Could you check a few things on this model? Use its own coordinates, in mm. Give positions to 0.01 mm unless a question says otherwise; leave off trailing zeros. Loops run counter-clockwise (first coordinate to the right, second up) from the corner with the lowest first, then second, coordinate; pieces in that order, holes last.
1. For P1, Ø1.5, axis at x = 37, y = 8, coming from the -Z side; P2, Ø8, axis at y = 23, z = -101.5, coming from the -X side; P3, Ø6, axis at x = 19.5, y = 24, coming from the -Z side, each with a flat end and sliding along its axis, tell me the tip position at first contact or that it passes through.
2. Thinking about a two-plate mould opening in Y: for faces 1 (the flat face through (36, 30, -13)), 2 (the flat face through (36, 0, -13)), 3 (the flat face through (148, 15, -182.326)), which applies, +Y half, -Y half, draft (parallel to the pull), parting line (faces both ways), or undercut?
3. Imagine slicing it at A-A (y = 15.75). List the corners of the cut face in (x, z) for me.
4. Imagine slicing it at B-B (z = -164.5). List the corners of the cut face in (x, y) for me.
5. I need wall thicknesses on line 1 along Z through (x, y) = (-13, 4); line 2 along X through (y, z) = (24.75, -147.5); line 3 along Z through (x, y) = (19.5, 22.75). Which ranges of each line are inside material? Lowest first, please.
6. Imagine slicing it at C-C (x = -41). List the corners of the cut face in (y, z) for me, plus the area to 3 significant figures.
```python
from build123d import *

# Parameters (mm, degrees)
EXTRUDE_1_DEPTH = 30


with BuildPart() as part:
    # 草图1 → 凸台-拉伸1 (new body)
    with BuildSketch(Plane(origin=(0, 0, 0), x_dir=(1, 0, 0), z_dir=(0, 1, 0))):
        Polygon((162.790697674, 182.325581395), (132.790697674, 182.325581395), (-87.209302326, 52.325581395), (-87.209302326, -97.674418605), (162.790697674, -97.674418605), align=None)
    extrude(amount=EXTRUDE_1_DEPTH)


solid = part.part
```
Derived:
1. P1: stops at z = -126.17
1. P2: stops at x = -10.76
1. P3: stops at z = -117.15
2. face 1: +Y half
2. face 2: -Y half
2. face 3: draft
3. outline: (-87.21, -52.33) - (132.79, -182.33) - (162.79, -182.33) - (162.79, 97.67) - (-87.21, 97.67) - close
4. outline: (102.62, 0) - (162.79, 0) - (162.79, 30) - (102.62, 30) - close
5. line 1: z = -96.18 to 97.67
5. line 2: x = 73.86 to 162.79
5. line 3: z = -115.38 to 97.67
6. outline: (0, -79.63) - (30, -79.63) - (30, 97.67) - (0, 97.67) - close
6. area: 5,320 mm2
